```python
from build123d import *

# Parameters (mm, degrees)
SKETCH1_W           = 200
SKETCH1_H           = 200
SKETCH1_W_2         = 151
SKETCH1_H_2         = 151
BOSS_EXTRUDE1_DEPTH = 20
FILLET1_R           = 20
FILLET2_R           = 10


with BuildPart() as part:
    # Sketch1 → Boss-Extrude1 (new body)
    with BuildSketch(Plane.XY):
        with Locations((100, 100)):
            Rectangle(SKETCH1_W, SKETCH1_H)
        with Locations((100, 100)):
            Rectangle(SKETCH1_W_2, SKETCH1_H_2, mode=Mode.SUBTRACT)
    extrude(amount=BOSS_EXTRUDE1_DEPTH)

    # Fillet1
    fillet1_edges = [part.edges().sort_by_distance(p)[0] for p in [
        (0, 200, 10),
        (200, 200, 10),
        (200, 0, 10),
        (0, 0, 10),
    ]]
    fillet(fillet1_edges, radius=FILLET1_R)

    # Fillet2
    fillet2_edges = [part.edges().sort_by_distance(p)[0] for p in [
        (24.5, 175.5, 10),
        (24.5, 24.5, 10),
        (175.5, 24.5, 10),
        (175.5, 175.5, 10),
    ]]
    fillet(fillet2_edges, radius=FILLET2_R)


solid = part.part
```
Could you check a few things on this model? Use its own coordinates, in mm. A direction names the side the tool comes from. Round coordinates to 2 decimals unless told otherwise and drop trailing zeros. Write each loop counter-clockwise with the first axis right and the second up, starting at its lowest first coordinate (ties: lowest second). Pieces come first, ordered by that corner, then holes. Notation, with made-up numbers: M 2.5,-22.75 L 23.5,-22.75 A16 ccw 23.5,-3.75 Z; hole C 71,37 d11. An arc over 180 degrees is marked long. Write each question's results on one line, items separated by ' | '. Start each with the question number.
1. I need wall thicknesses on L1, parallel to X at y = 83.5, z = 10.75; L2, parallel to Y at x = 172, z = 7.5. Which ranges of each line are inside material? Lowest first, please. Write a range as from..to.
2. On a 3-axis mill with a long thin cutter (end or side, diameter ignored), from which of +Z, -Z, +X, -X, +Y, -Y can I reach the whole of each face in a straight line? I mean faces 4 (the face through (24.5, 99, 10)), 5 (the face through (200, 99, 10)). Say none if no direction works.
3. Imagine slicing it at B-B on z = 12.25. List the corners of the cut face in (x, y) for me, and give its area (3 significant figures).
4. Imagine slicing it at A-A on y = 64. List the corners of the cut face in (x, z) for me, and give its area (3 significant figures).
5. Thinking about a two-plate mould opening in X: for faces 1 (the face through (175.5, 99, 10)), 2 (the face through (99, 0, 10)), 3 (the face through (193.986, 194.297, 10.14)), which applies, +X half, -X half, draft (parallel to the pull), parting line (faces both ways), or undercut?
Result sheet:
1) L1: x = 0..24.5, 175.5..200 | L2: y = 0..26.9, 173.1..200
2) face 4: +Z, -Z | face 5: +Z, -Z, +X, +Y, -Y
3) outline: M 0,20 A20 ccw 20,0 L 180,0 A20 ccw 200,20 L 200,180 A20 ccw 180,200 L 20,200 A20 ccw 0,180 Z; hole M 24.5,34.5 A10 ccw 34.5,24.5 L 165.5,24.5 A10 ccw 175.5,34.5 L 175.5,165.5 A10 ccw 165.5,175.5 L 34.5,175.5 A10 ccw 24.5,165.5 Z | area: 16,900 mm^2
4) outline: M 0,0 L 24.5,0 L 24.5,20 L 0,20 Z; M 175.5,0 L 200,0 L 200,20 L 175.5,20 Z | area: 980 mm^2
5) face 1: undercut | face 2: draft | face 3: +X half
